```python
from build123d import *

# Parameters (mm, degrees)
BASE_PLATE_DEPTH         = 12
SIDE_FLANGE_DEPTH        = 12
BOSS_88MM_DEPTH          = 88
CURVED_START             = -12
CURVED_CUT_DEPTH         = 12
SLOT_A_SKETCH_22_5X7_5_W = 25
SLOT_A_SKETCH_22_5X7_5_H = 15
SLOT_A_22_5X7_5_DEPTH    = 12
SLOT_B_SKETCH_7_5X22_5_W = 25
SLOT_B_SKETCH_7_5X22_5_H = 15
SLOT_B_7_5X22_5_DEPTH    = 12
HOLE_A_SKETCH_15_R       = 7.5
HOLE_A_15_DEPTH          = 12
HOLE_B_SKETCH_15_R       = 7.5
HOLE_B_15_DEPTH          = 12


with BuildPart() as part:
    # Base Plate Sketch → Base Plate (new body)
    with BuildSketch(Plane.XY):
        with BuildLine():
            Line((0, 0), (0, -75))
            ThreePointArc((0, -75), (7.32233047, -92.67766953), (25, -100))
            Line((25, -100), (115, -100))
            ThreePointArc((115, -100), (132.67766953, -92.67766953), (140, -75))
            Line((140, -75), (140, 0))
            Line((140, 0), (0, 0))
        make_face()
    extrude(amount=BASE_PLATE_DEPTH)

    # Side Flange Sketch → Side Flange (add)
    with BuildSketch(Plane(origin=(0, 0, 0), x_dir=(1, 0, 0), z_dir=(0, 1, 0))):
        with BuildLine():
            Line((140, -12), (140, -47))
            ThreePointArc((140, -47), (132.67766953, -64.67766953), (115, -72))
            Line((115, -72), (25, -72))
            ThreePointArc((25, -72), (7.32233047, -64.67766953), (0, -47))
            Line((0, -47), (0, -12))
            Line((0, -12), (140, -12))
        make_face()
    extrude(amount=-SIDE_FLANGE_DEPTH)

    # Boss Profile Sketch → Boss 88mm (add)
    with BuildSketch(Plane.XZ.offset(12)):
        with BuildLine():
            Line((95, 72), (100, 72))
            Line((100, 72), (100, 12))
            Line((100, 12), (40, 12))
            Line((40, 12), (40, 72))
            Line((40, 72), (45, 72))
            ThreePointArc((45, 72), (70, 47), (95, 72))
        make_face()
    extrude(amount=BOSS_88MM_DEPTH)

    # Curved Cut Sketch → Curved Cut (cut)
    with BuildSketch(Plane.XZ.offset(12).offset(CURVED_START)):
        with BuildLine():
            Line((45, 72), (95, 72))
            ThreePointArc((95, 72), (70, 47), (45, 72))
        make_face()
    extrude(amount=CURVED_CUT_DEPTH, mode=Mode.SUBTRACT)

    # Slot A Sketch 22.5x7.5 → Slot A 22.5x7.5 (cut)
    with BuildSketch(Plane(origin=(0, -12, 0), x_dir=(-1, 0, 0), z_dir=(0, -1, 0))):
        with Locations((-120, -42)):
            Rectangle(SLOT_A_SKETCH_22_5X7_5_W, SLOT_A_SKETCH_22_5X7_5_H)
    extrude(amount=-SLOT_A_22_5X7_5_DEPTH, mode=Mode.SUBTRACT)

    # Slot B Sketch 7.5x22.5 → Slot B 7.5x22.5 (cut)
    with BuildSketch(Plane(origin=(0, -12, 0), x_dir=(-1, 0, 0), z_dir=(0, -1, 0))):
        with Locations((-20, -42)):
            Rectangle(SLOT_B_SKETCH_7_5X22_5_W, SLOT_B_SKETCH_7_5X22_5_H)
    extrude(amount=-SLOT_B_7_5X22_5_DEPTH, mode=Mode.SUBTRACT)

    # Hole A Sketch Ø15 → Hole A Ø15 (cut)
    with BuildSketch(Plane.XY.offset(12)):
        with Locations((119.463154548, -27)):
            Circle(HOLE_A_SKETCH_15_R)
        with Locations((119.463154548, -77)):
            Circle(HOLE_A_SKETCH_15_R)
    extrude(amount=-HOLE_A_15_DEPTH, mode=Mode.SUBTRACT)

    # Hole B Sketch Ø15 → Hole B Ø15 (cut)
    with BuildSketch(Plane.XY.offset(12)):
        with Locations((19.128084721, -27)):
            Circle(HOLE_B_SKETCH_15_R)
        with Locations((19.128084721, -77)):
            Circle(HOLE_B_SKETCH_15_R)
    extrude(amount=-HOLE_B_15_DEPTH, mode=Mode.SUBTRACT)


solid = part.part
```
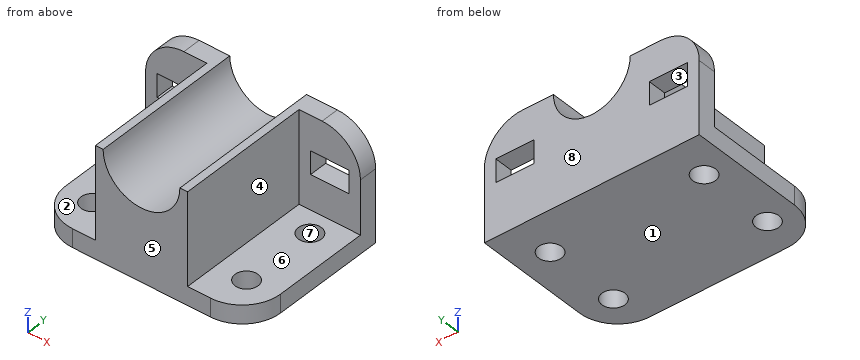
Here's how the part is built. I have some questions about the finished solid (model axes, mm). Face numbers are marked on the shaded views. A direction names the side the tool comes from. Coordinates: 2 decimals unless noted, no trailing zeros. Loops run counter-clockwise (first coordinate to the right, second up) from the corner with the lowest first, then second, coordinate; pieces in that order, holes last. Notation, with made-up numbers: (43.5, 52.5) - (94.5, 52.5) arc R34 ccw to (94.5, 85.5) - close; hole circle Ø3 at (24.5, -21.5). An arc over 180 degrees is marked (long way). Return JSON: item names as keys, results as strings. Group by question number.
Item 1: I need wall thicknesses on line 1 (Y direction, x = 35.5, z = 29.5); line 2 (Z direction, x = 70.5, y = -90) (3 decimals); line 3 (Z direction, x = 105, y = -21). Which ranges of each line are inside material? Lowest first, please. Write a range as from..to.
Item 2: Will these pins go through, and if not, where does the flat tip stop? P1, Ø20, axis at x = 11, y = -77, coming from the +Z side; P2, Ø10, axis at y = -69, z = 57.5, coming from the +X side; P3, Ø1, axis at y = -61, z = 58.5, coming from the -X side.
Item 3: If we section it at C-C on y = -27: Write out the boundary of the cut face in (x, z), and give its area (3 significant figures).
Item 4: On a 3-axis mill with a long thin cutter (end or side, diameter ignored), from which of +Z, -Z, +X, -X, +Y, -Y can I reach the whole of each face in a straight line? I mean the marked faces 1, 2, 3, 4 and 5. Say none if no direction works.
Item 5: If we section it at A-A on y = -7: Write out the boundary of the cut face in (x, z), and give its area (3 significant figures).
Item 6: We'd pull the mould along Y, two halves only. Please class the marked faces 6, 7 and 8: +Y half, -Y half, draft (parallel to the pull), parting line (faces both ways), or undercut.
Item 7: If we section it at B-B on z = 42.5: Write out the boundary of the cut face in (x, y).
Item 8: If we section it at D-D on x = 104: Write out the boundary of the cut face in (y, z).
Calculated:
{
 "1": {"line 1": "y = -12..0", "line 2": "z = 0..47.005", "line 3": "z = 0..12"},
 "2": {"P1": "stops at z = 12", "P2": "stops at x = 100", "P3": "stops at x = 40"},
 "3": {"outline": "(0, 0) - (11.63, 0) - (11.63, 12) - (0, 12) - close; (26.63, 0) - (111.96, 0) - (111.96, 12) - (100, 12) - (100, 72) - (95, 72) arc R25 cw to (45, 72) - (40, 72) - (40, 12) - (26.63, 12) - close; (126.96, 0) - (140, 0) - (140, 12) - (126.96, 12) - close", "area": "3,940 mm^2"},
 "4": {"face 1": "-Z, +X, -X, +Y, -Y", "face 2": "+Z, -X, -Y", "face 3": "+Y, -Y", "face 4": "+Z, +X, -Y", "face 5": "+Z, -Z, +X, -X, -Y"},
 "5": {"outline": "(0, 0) - (140, 0) - (140, 47) arc R25 ccw to (115, 72) - (95, 72) arc R25 cw to (45, 72) - (25, 72) arc R25 ccw to (0, 47) - close; hole (7.5, 34.5) - (32.5, 34.5) - (32.5, 49.5) - (7.5, 49.5) - close; hole (107.5, 34.5) - (132.5, 34.5) - (132.5, 49.5) - (107.5, 49.5) - close", "area": "8,080 mm^2"},
 "6": {"face 6": "draft", "face 7": "undercut", "face 8": "+Y half"},
 "7": {"outline": "(0, -12) - (7.5, -12) - (7.5, 0) - (0, 0) - close; (32.5, -12) - (40, -12) - (40, -100) - (100, -100) - (100, -12) - (107.5, -12) - (107.5, 0) - (32.5, 0) - close; (132.5, -12) - (140, -12) - (140, 0) - (132.5, 0) - close"},
 "8": {"outline": "(-100, 0) - (0, 0) - (0, 72) - (-12, 72) - (-12, 12) - (-100, 12) - close"}
}
